Can you work these out from the drawing? Everything is in mm from the part's minimum corner. A direction names the side the tool comes from. Round coordinates to 2 decimals unless told otherwise and drop trailing zeros. Loops run counter-clockwise (first coordinate to the right, second up) from the corner with the lowest first, then second, coordinate; pieces in that order, holes last. Notation, with made-up numbers: M -39.75,10.25 L -33.75,10.25 A27 cw -33.75,49.25 Z; hole C 54,-24.75 d10. An arc over 180 degrees is marked long. Return JSON: item names as keys, results as strings. Group by question number.
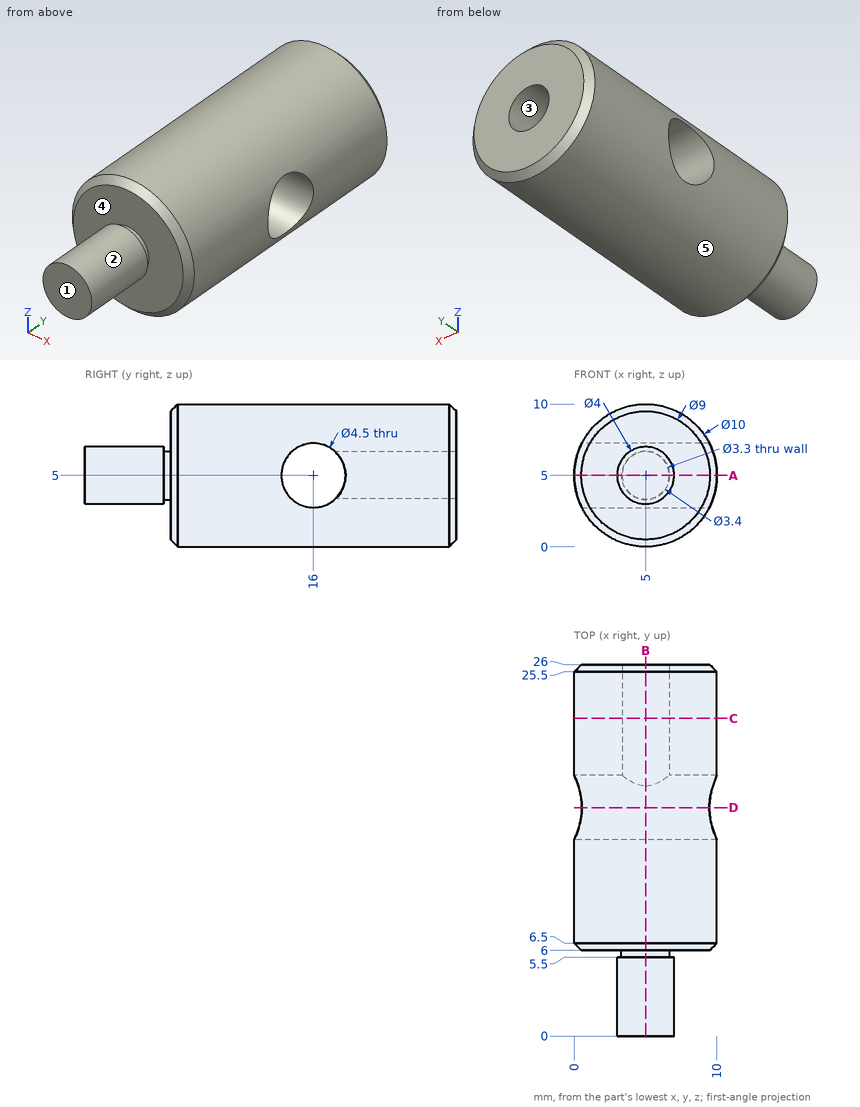
1. I need wall thicknesses on probe 1 along Z at (x, y) = (4.75, 16); probe 2 along Z at (x, y) = (4, 15.25); probe 3 along Y at (x, z) = (3.25, 1.75). Which ranges of each line are inside material? Lowest first, please.
2. If we section it at A-A, the plane z = 5: Please give me the cut outline in (x, y).
3. If we section it at D-D, the plane y = 16: Please give me the cut outline in (x, z).
4. I'm going to push flat-ended pins straight in: pin 1 Ø2.5 at (x, z) = (4, 3.5) entering from -Y; pin 2 Ø1.5 at (y, z) = (17, 3) entering from +X; pin 3 Ø6 at (x, y) = (8.5, 20.5) entering from -Z; pin 4 Ø1 at (x, y) = (1.5, 22) entering from -Z. Where does each tip first touch, or does it pass through?
5. We'd pull the mould along X, two halves only. Please class the marked faces 3, 4 and 5: +X half, -X half, draft (parallel to the pull), parting line (faces both ways), or undercut.
6. If we section it at B-B, the plane x = 5: Please give me the cut outline in (y, z).
7. On a 3-axis mill with a long thin cutter (end or side, diameter ignored), from which of +Z, -Z, +X, -X, +Y, -Y can I reach the whole of each face in a straight line? I mean the marked faces 1 and 2. Say none if no direction works.
8. If we section it at C-C, the plane y = 22.25: Please give me the cut outline in (x, z), then the cut area to 3 significant figures.
Geometry results:
{
 "1": {"probe 1": "0.01 to 2.75, 7.25 to 9.99", "probe 2": "0.1 to 2.88, 7.12 to 9.9", "probe 3": "6 to 26"},
 "2": {"outline": "M 0,6.5 L 0.5,6 L 3.3,6 L 3.3,5.5 L 3,5.5 L 3,0 L 7,0 L 7,5.5 L 6.7,5.5 L 6.7,6 L 9.5,6 L 10,6.5 L 10,13.75 L 0,13.75 Z; M 0,18.25 L 3.35,18.25 L 3.35,26 L 0.5,26 L 0,25.5 Z; M 6.65,18.25 L 10,18.25 L 10,25.5 L 9.5,26 L 6.65,26 Z"},
 "3": {"outline": "M 0.53,2.75 A5 ccw 9.47,2.75 Z; M 0.53,7.25 L 9.47,7.25 A5 ccw Z"},
 "4": {"pin 1": "y = 0", "pin 2": "x = 9.75", "pin 3": "z = 0.03", "pin 4": "z = 1"},
 "5": {"face 3": "undercut", "face 4": "draft", "face 5": "parting line"},
 "6": {"outline": "M 0,3 L 5.5,3 L 5.5,3.3 L 6,3.3 L 6,0.5 L 6.5,0 L 25.5,0 L 26,0.5 L 26,3.35 L 17.53,3.35 A2.25 cw long 17.53,6.65 L 26,6.65 L 26,9.5 L 25.5,10 L 6.5,10 L 6,9.5 L 6,6.7 L 5.5,6.7 L 5.5,7 L 0,7 Z"},
 "7": {"face 1": "+Z, -Z, +X, -X, -Y", "face 2": "-Y"},
 "8": {"outline": "C 5,5 d10; hole C 5,5 d3.3", "area": "70.0 mm^2"}
}
